Here's the drawing with two shaded views (mm, measured from the low corner). I have some questions. A direction names the side the tool comes from. Coordinates: 2 decimals unless noted, no trailing zeros. Order: outer loops, then holes, each group sorted by start corner. A loop starts at its lowest first (then second) coordinate and runs counter-clockwise, first axis right, second up. Notation, with made-up numbers: (-18, 63) -> (-9, 63) arc R13 ccw to (-9, 77) -> close; hole circle Ø10 at (-13, -33). An arc over 180 degrees is marked (long way). Answer in a Markdown table with one row per item. Add a question column.
1. Imagine slicing it at C-C on x = 53. Write out the boundary of the cut face in (y, z), plus the area to 3 significant figures.
2. Will these pins go through, and if not, where does the flat tip stop? pin 1 (7 mm diameter, centred on x = 422.5, z = 215.5, fed in from -Y); pin 2 (13 mm diameter, centred on x = 157.5, z = 32.5, fed in from +Y); pin 3 (15 mm diameter, centred on x = 555, z = 215.5, fed in from -Y); pin 4 (5 mm diameter, centred on x = 311, y = 5.5, fed in from +Z).
3. If I drill on line 1 along X through (y, z) = (24.5, 215.5); line 2 along Z through (x, y) = (555, 24); line 3 along X through (y, z) = (16, 213), over which ranges is the centre line in solid material (lowest first)? Write a range as [from, to].
4. Imagine slicing it at B-B on z = 32.5. State how many separate pieces and enclosed holes the cut face has, plus the area to 3 significant figures.
5. On a 3-axis mill with a long thin cutter (end or side, diameter ignored), from which of +Z, -Z, +X, -X, +Y, -Y can I reach the whole of each face in a straight line? I mean the marked faces 1 and 2. Say none if no direction works.
6. Imagine slicing it at A-A on x = 422.5. Write out the boundary of the cut face in (y, z), plus the area to 3 significant figures.
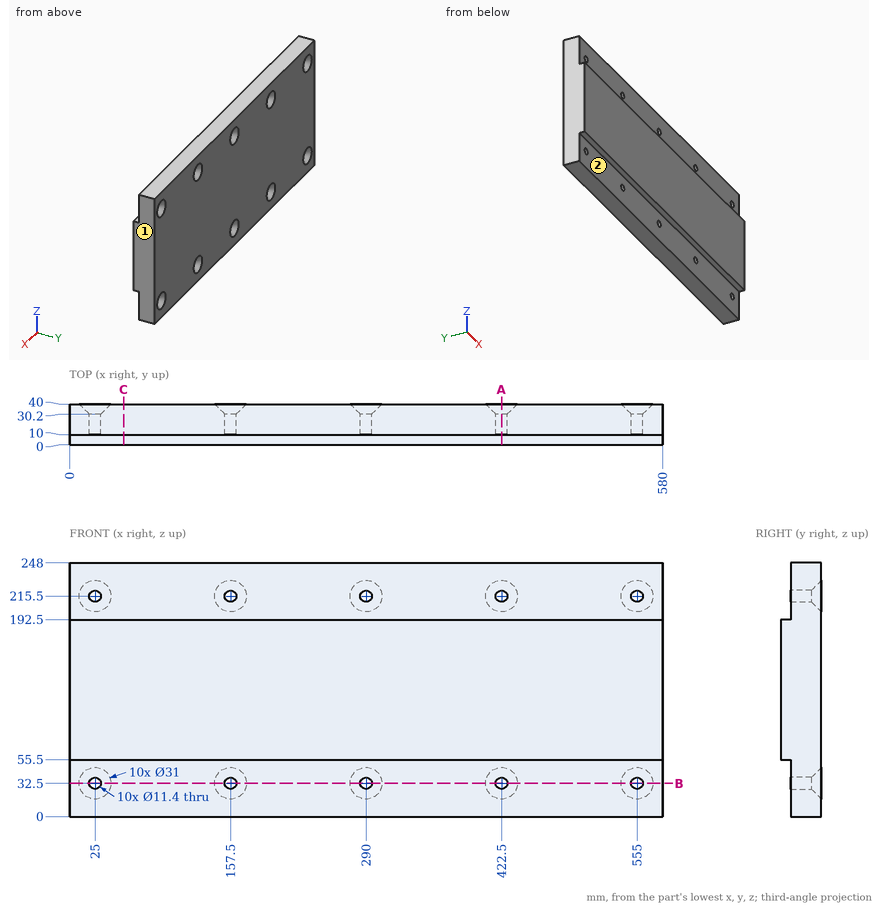
Answers follow:
| question | item | result |
|---|---|---|
| 1 | outline | (0, 55.5) -> (10, 55.5) -> (10, 0) -> (40, 0) -> (40, 248) -> (10, 248) -> (10, 192.5) -> (0, 192.5) -> close |
| 1 | area | 8,810 mm² |
| 2 | pin 1 | passes through |
| 2 | pin 2 | stops at y = 31 |
| 2 | pin 3 | stops at y = 10 |
| 2 | pin 4 | stops at z = 192.5 |
| 3 | line 1 | x = [0, 19.3], [30.7, 151.8], [163.2, 284.3], [295.7, 416.8], [428.2, 549.3], [560.7, 580] |
| 3 | line 2 | z = [0, 26.8], [38.2, 209.8], [221.2, 248] |
| 3 | line 3 | x = [0, 19.88], [30.12, 152.38], [162.62, 284.88], [295.12, 417.38], [427.62, 549.88], [560.12, 580] |
| 4 | separate pieces | 6 |
| 4 | enclosed holes | 0 |
| 4 | area | 15,200 mm² |
| 5 | face 1 | +Z, -Z, +X, +Y, -Y |
| 5 | face 2 | -Z, +X, -X, -Y |
| 6 | outline | (0, 55.5) -> (10, 55.5) -> (10, 38.2) -> (30.2, 38.2) -> (40, 48) -> (40, 200) -> (30.2, 209.8) -> (10, 209.8) -> (10, 192.5) -> (0, 192.5) -> close; (10, 0) -> (40, 0) -> (40, 17) -> (30.2, 26.8) -> (10, 26.8) -> close; (10, 221.2) -> (30.2, 221.2) -> (40, 231) -> (40, 248) -> (10, 248) -> close |
| 6 | area | 7,930 mm² |
